Design review of the part built by this model. Coordinates are the model's own, in mm. A direction names the side the tool comes from. Round coordinates to 2 decimals unless told otherwise and drop trailing zeros. Order: outer loops, then holes, each group sorted by start corner. A loop starts at its lowest first (then second) coordinate and runs counter-clockwise, first axis right, second up. Notation, with made-up numbers: M -24.5,23.25 L -11.5,23.25 A6 cw -11.5,32.25 Z; hole C 17.5,58 d11. An arc over 180 degrees is marked long. Use a Markdown table: item, result. Add a question column.
(1) Take a section at A-A (x = -30). Write out the cut boundary in (y, z).
(2) To check wall thickness, follow probe 1 along X at (y, z) = (1, 0); probe 2 along X at (y, z) = (1.4, -45); probe 3 along Z at (x, y) = (17, 3.15). State the ranges of each line that lie inside material, in increasing order. Write a range as from..to.
(3) For pin 1 (10 mm diameter, centred on x = -15.5, z = -18, fed in from -Y); pin 2 (2.5 mm diameter, centred on x = -4, y = 1.5, fed in from -Z); pin 3 (2.5 mm diameter, centred on y = 3, z = -30, fed in from +X), all flat-tipped, find the tip position at first contact; note any pin that passes through.
(4) Machinability: for faces 1 (the face through (-5, 2, 5)), 2 (the face through (0, 2, -5)), which of the approach directions +Z, -Z, +X, -X, +Y, -Y give a long, thin tool a straight path to every point of the face, cutting with its end or side? Answer none if there is none.
(5) Take a section at C-C (z = 0). Write out the cut boundary in (x, y).
(6) Take a section at D-D (z = -13). Write out the cut boundary in (x, y), then the cut area to 3 significant figures.
(7) Take a section at B-B (y = 1.3). Write out the cut boundary in (x, z).
(8) The part is to be moulded in two halves that separate along Z. For faces 3 (the face through (27.48, 2.46, -0.33)), 4 (the face through (-25, 2, -25)), 5 (the face through (-30, 2, -50)), 6 (the face through (-27.89, 2.46, -43.66)), say which applies: released by +Z, released by -Z, zero draft, split by the parting line, or undercut.
```python
from build123d import *

# Parameters (mm, degrees)
SKETCH1_R           = 2.5
BOSS_EXTRUDE1_DEPTH = 5


with BuildPart() as part:
    # Sketch1 → Boss-Extrude1 (new body)
    with BuildSketch(Plane(origin=(0, 0, 0), x_dir=(1, 0, 0), z_dir=(0, 1, 0))):
        with BuildLine():
            Line((-25, -5), (25, -5))
            ThreePointArc((25, -5), (30, 0), (25, 5))
            Line((25, 5), (-25, 5))
            Line((-25, 5), (-25, 45))
            ThreePointArc((-25, 45), (-30, 50), (-35, 45))
            Line((-35, 45), (-35, -5))
            Line((-35, -5), (-25, -5))
        make_face()
        with Locations(Location((25, 0, 0), (0, 0, 270))):
            Circle(SKETCH1_R, mode=Mode.SUBTRACT)
        with Locations(Location((-30, 45, 0), (0, 0, 270))):
            Circle(SKETCH1_R, mode=Mode.SUBTRACT)
    extrude(amount=BOSS_EXTRUDE1_DEPTH)


solid = part.part
```
Verdict:
| question | item | result |
|---|---|---|
| 1 | outline | M 0,-50 L 5,-50 L 5,-47.5 L 0,-47.5 Z; M 0,-42.5 L 5,-42.5 L 5,5 L 0,5 Z |
| 2 | probe 1 | x = -35..22.5, 27.5..30 |
| 2 | probe 2 | x = -35..-32.5, -27.5..-25 |
| 2 | probe 3 | z = -5..5 |
| 3 | pin 1 | passes through |
| 3 | pin 2 | stops at z = -5 |
| 3 | pin 3 | stops at x = -25 |
| 4 | face 1 | +Z, +X, -X, +Y, -Y |
| 4 | face 2 | -Z, +X, +Y, -Y |
| 5 | outline | M -35,0 L 22.5,0 L 22.5,5 L -35,5 Z; M 27.5,0 L 30,0 L 30,5 L 27.5,5 Z |
| 6 | outline | M -35,0 L -25,0 L -25,5 L -35,5 Z |
| 6 | area | 50.0 mm^2 |
| 7 | outline | M -35,-45 A5 ccw -25,-45 L -25,-5 L 25,-5 A5 ccw 25,5 L -35,5 Z; hole C -30,-45 d5; hole C 25,0 d5 |
| 8 | face 3 | undercut |
| 8 | face 4 | zero draft |
| 8 | face 5 | released by -Z |
| 8 | face 6 | undercut |
